```python
from build123d import *

# Parameters (mm, degrees)
BOSS_EXTRUDE1_DEPTH = 915


with BuildPart() as part:
    # Sketch1 → Boss-Extrude1 (new body)
    with BuildSketch(Plane(origin=(-422.5, 0, 0), x_dir=(0, -1, 0), z_dir=(-1, 0, 0))):
        with BuildLine():
            Line((-755.11, 454.95), (-755.11, 452.15))
            ThreePointArc((-755.11, 452.15), (-755.183223305, 451.973223305), (-755.36, 451.9))
            Line((-755.36, 451.9), (-762.01, 451.9))
            Line((-762.01, 451.9), (-762.01, 452.7))
            Line((-762.01, 452.7), (-762.56, 452.7))
            ThreePointArc((-762.56, 452.7), (-762.736776695, 452.626776695), (-762.81, 452.45))
            Line((-762.81, 452.45), (-762.81, 451.35))
            ThreePointArc((-762.81, 451.35), (-762.736776695, 451.173223305), (-762.56, 451.1))
            Line((-762.56, 451.1), (-755.31, 451.1))
            ThreePointArc((-755.31, 451.1), (-754.602893219, 451.392893219), (-754.31, 452.1))
            Line((-754.31, 452.1), (-754.31, 453.373491886))
            ThreePointArc((-754.31, 453.373491886), (-753.775028159, 454.665028159), (-752.483491886, 455.2))
            Line((-752.483491886, 455.2), (-752.41, 455.2))
            ThreePointArc((-752.41, 455.2), (-751.702893219, 455.492893219), (-751.41, 456.2))
            Line((-751.41, 456.2), (-751.41, 458.6))
            ThreePointArc((-751.41, 458.6), (-751.849339828, 459.660660172), (-752.91, 460.1))
            Line((-752.91, 460.1), (-753.31, 460.1))
            ThreePointArc((-753.31, 460.1), (-754.301183271, 459.232498012), (-753.572659626, 458.135111446))
            Line((-753.572659626, 458.135111446), (-752.947340374, 457.964888554))
            ThreePointArc((-752.947340374, 457.964888554), (-752.218816729, 456.867501988), (-753.21, 456))
            Line((-753.21, 456), (-768.909810447, 456))
            ThreePointArc((-768.909810447, 456), (-769.900988627, 456.867463908), (-769.172544211, 457.964868369))
            Line((-769.172544211, 457.964868369), (-768.547266236, 458.135131631))
            ThreePointArc((-768.547266236, 458.135131631), (-767.81882182, 459.232536092), (-768.81, 460.1))
            Line((-768.81, 460.1), (-769.21, 460.1))
            ThreePointArc((-769.21, 460.1), (-770.270660172, 459.660660172), (-770.71, 458.6))
            Line((-770.71, 458.6), (-770.71, 456))
            ThreePointArc((-770.71, 456), (-770.959658895, 455.534896264), (-771.353431907, 455.183337075))
            ThreePointArc((-771.353431907, 455.183337075), (-771.39533621, 455.130932577), (-771.394682745, 455.06383731))
            ThreePointArc((-771.394682745, 455.06383731), (-771.317838721, 454.956126495), (-771.196783129, 454.902720811))
            ThreePointArc((-771.196783129, 454.902720811), (-771.165207963, 454.903064362), (-771.135314114, 454.913236231))
            ThreePointArc((-771.135314114, 454.913236231), (-770.541156786, 455.135665686), (-769.91, 455.2))
            Line((-769.91, 455.2), (-755.36, 455.2))
            ThreePointArc((-755.36, 455.2), (-755.183223305, 455.126776695), (-755.11, 454.95))
        make_face()
    extrude(amount=-BOSS_EXTRUDE1_DEPTH)


solid = part.part
```
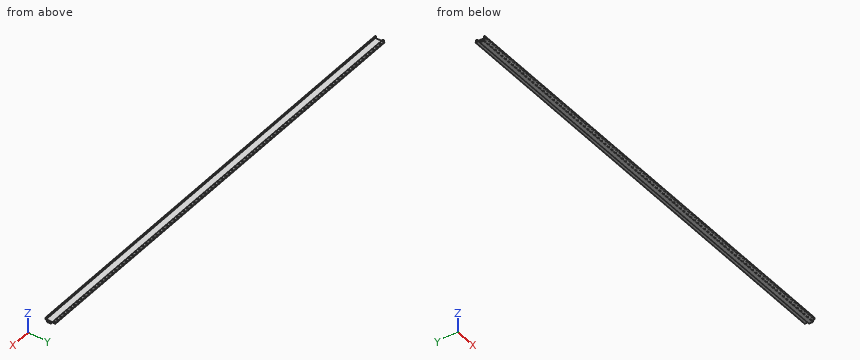
Input: part model. Units: mm. Frame: model coordinates. Give positions to 0.01 mm unless a question says otherwise; leave off trailing zeros. Order: outer loops, then holes, each group sorted by start corner. A loop starts at its lowest first (then second) coordinate and runs counter-clockwise, first axis right, second up.
1. Pin query (flat end, axial travel): pin 1 Ø3.5 at (x, y) = (128, 759.5) entering from +Z; pin 2 Ø10 at (x, y) = (-66.5, 765.5) entering from -Z; pin 3 Ø1.2 at (x, z) = (255, 452) entering from +Y; pin 4 Ø1.5 at (y, z) = (765, 457.5) entering from -X. Return the tip coordinate at first contact, or that it passes through.
Computed:
pin 1: stops at z = 456
pin 2: stops at z = 451.1
pin 3: stops at y = 762.81
pin 4: passes through
2. Cut plane A-A (y = 758.5). Return loops of the section in (x, z).
Computed:
outline: (-422.5, 451.1) - (492.5, 451.1) - (492.5, 451.9) - (-422.5, 451.9) - close; (-422.5, 455.2) - (492.5, 455.2) - (492.5, 456) - (-422.5, 456) - close
3. Line query: probe 1 along Y at (x, z) = (151, 456.5); probe 2 along Y at (x, z) = (225, 455); probe 3 along Z at (x, y) = (388.5, 759). Output: solid intervals per line, ascending.
Computed:
probe 1: y = 751.41 to 752.34, 769.78 to 770.71
probe 2: y = 753.31 to 755.12, 770.95 to 771.36
probe 3: z = 451.1 to 451.9, 455.2 to 456
